```python
from build123d import *

# Parameters (mm, degrees)
CHAMFER_1_SIZE  = 1
CHAMFER_1_SIZE2 = 1.414213562
EXTRUDE_1_DEPTH = 15
EXTRUDE_2_DEPTH = 35
CHAMFER_2_SIZE  = 8


with BuildPart() as part:
    # 草图1 → 旋转1 (revolve)
    with BuildSketch(Plane.XY, mode=Mode.PRIVATE) as revolve_1_sk:
        Polygon((0, 0), (35, 0), (35, 10), (26.961524227, 40), (0, 40), align=None)
    revolve(revolve_1_sk.sketch.rotate(Axis((0, 40, 0), (0, -1, 0)), 180), axis=Axis((0, 40, 0), (0, -1, 0)))

    # 倒角1
    chamfer_1_edges = [part.edges().sort_by_distance(p)[0] for p in [
        (26.961524227, 40, 0),
    ]]
    chamfer_1_side = [part.faces().sort_by_distance(p)[0] for p in [
        (30.980762114, 25, 0),
    ]]
    chamfer(chamfer_1_edges, length=CHAMFER_1_SIZE, length2=CHAMFER_1_SIZE2, reference=chamfer_1_side[0])

    # 草图2 → 凸台-拉伸1 (add)
    with BuildSketch(Plane.XZ):
        with BuildLine():
            Line((44, -60), (-44, -60))
            ThreePointArc((-44, -60), (-55.313708499, -55.313708499), (-60, -44))
            Line((-60, -44), (-60, 44))
            ThreePointArc((-60, 44), (-55.313708499, 55.313708499), (-44, 60))
            Line((-44, 60), (44, 60))
            ThreePointArc((44, 60), (55.313708499, 55.313708499), (60, 44))
            Line((60, 44), (60, -44))
            ThreePointArc((60, -44), (55.313708499, -55.313708499), (44, -60))
        make_face()
    extrude(amount=EXTRUDE_1_DEPTH)

    # 草图3 → 凸台-拉伸2 (add)
    with BuildSketch(Plane.XZ.offset(15)):
        with BuildLine():
            Line((36, -50), (-36, -50))
            ThreePointArc((-36, -50), (-45.899494937, -45.899494937), (-50, -36))
            Line((-50, -36), (-50, 36))
            ThreePointArc((-50, 36), (-45.899494937, 45.899494937), (-36, 50))
            Line((-36, 50), (36, 50))
            ThreePointArc((36, 50), (45.899494937, 45.899494937), (50, 36))
            Line((50, 36), (50, -36))
            ThreePointArc((50, -36), (45.899494937, -45.899494937), (36, -50))
        make_face()
    extrude(amount=EXTRUDE_2_DEPTH)

    # 倒角2
    chamfer_2_edges = [part.edges().sort_by_distance(p)[0] for p in [
        (-55.313708499, -15, -55.313708499),
        (0, -15, -60),
        (55.313708499, -15, -55.313708499),
        (60, -15, 0),
        (55.313708499, -15, 55.313708499),
        (0, -15, 60),
        (-55.313708499, -15, 55.313708499),
        (-60, -15, 0),
    ]]
    chamfer(chamfer_2_edges, length=CHAMFER_2_SIZE)


solid = part.part
```
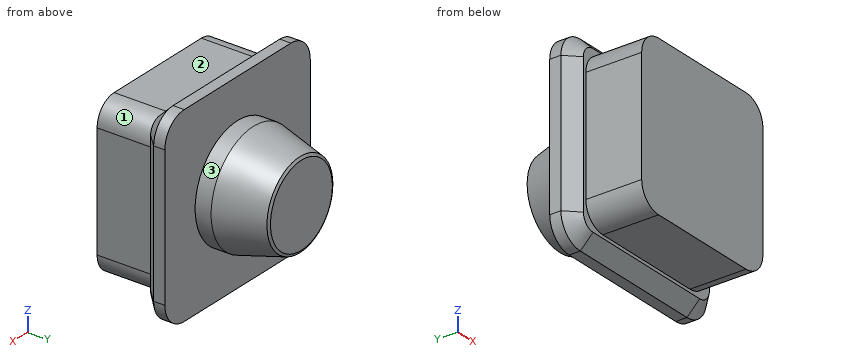
Could you check a few things on this model? Use its own coordinates, in mm. Face numbers are marked on the shaded views. A direction names the side the tool comes from. Round coordinates to 2 decimals unless told otherwise and drop trailing zeros. Loops run counter-clockwise (first coordinate to the right, second up) from the corner with the lowest first, then second, coordinate; pieces in that order, holes last. Notation, with made-up numbers: M 17,67.25 L 62,67.25 A8 cw 62,77.25 Z; hole C 74,-4 d1. An arc over 180 degrees is marked long. Put each result on its own line as item: value.
Q1. Imagine slicing it at D-D (y = 30). Write out the boundary of the cut face in (x, z), then the cut area to 3 significant figures.
Check result:
outline: C 0,0 d59.28
area: 2,760 mm2
Q2. For pin 1 (10 mm diameter, centred on y = -23.5, z = 31, fed in from +X); pin 2 (12 mm diameter, centred on y = 26.5, z = -17.5, fed in from -X); pin 3 (6 mm diameter, centred on x = 32.5, y = -30.5, fed in from +Z), each with a flat end and sliding along its axis, tell me the tip position at first contact or that it passes through.
Check result:
pin 1: x = 50
pin 2: x = -28.88
pin 3: z = 50
Q3. Imagine slicing it at A-A (x = 0). Write out the boundary of the cut face in (y, z).
Check result:
outline: M -50,-50 L -15,-50 L -15,-52 L -7,-60 L 0,-60 L 0,-35 L 10,-35 L 39.03,-27.22 L 40,-25.55 L 40,25.55 L 39.03,27.22 L 10,35 L 0,35 L 0,60 L -7,60 L -15,52 L -15,50 L -50,50 Z
Q4. Imagine slicing it at B-B (z = 0). Write out the boundary of the cut face in (x, y), then the cut area to 3 significant figures.
Check result:
outline: M -60,-7 L -52,-15 L -50,-15 L -50,-50 L 50,-50 L 50,-15 L 52,-15 L 60,-7 L 60,0 L 35,0 L 35,10 L 27.22,39.03 L 25.55,40 L -25.55,40 L -27.22,39.03 L -35,10 L -35,0 L -60,0 Z
area: 7,790 mm2
Q5. I need wall thicknesses on probe 1 along X at (y, z) = (-28, -3); probe 2 along Z at (x, y) = (37, -45); probe 3 along Y at (x, z) = (-42, 35). Which ranges of each line are inside material? Lowest first, please.
Check result:
probe 1: -50 to 50
probe 2: -49.96 to 49.96
probe 3: -50 to 0
Q6. On a 3-axis mill with a long thin cutter (end or side, diameter ignored), from which of +Z, -Z, +X, -X, +Y, -Y can I reach the whole of each face in a straight line? I mean the marked faces 1, 2 and 3. Say none if no direction works.
Check result:
face 1: +Z, +X, -Y
face 2: +Z, +X, -X, -Y
face 3: +Y
Q7. Imagine slicing it at C-C (y = -21). Write out the boundary of the cut face in (x, z).
Check result:
outline: M -50,-36 A14 ccw -36,-50 L 36,-50 A14 ccw 50,-36 L 50,36 A14 ccw 36,50 L -36,50 A14 ccw -50,36 Z
